from build123d import *

# Parameters (mm, degrees)
PATTERN_LINEAR_1_COUNT      = 2
PATTERN_LINEAR_1_PITCH      = 30.405591591
PATTERN_LINEAR_1_COUNT_DIR2 = 2
PATTERN_LINEAR_1_PITCH_DIR2 = 30.405591591


with BuildPart() as part:
    # 草图1 → 旋转1 (revolve)
    with BuildSketch(Plane.XY, mode=Mode.PRIVATE) as revolve_1_sk:
        with BuildLine():
            Line((0, 27), (0, 10))
            Line((0, 10), (65, 10))
            Line((65, 10), (65, 14.4))
            ThreePointArc((65, 14.4), (64.53137085, 15.53137085), (63.4, 16))
            Line((63.4, 16), (9.5, 16))
            Line((9.5, 16), (9.5, 15.5))
            Line((9.5, 15.5), (8, 15.5))
            Line((8, 15.5), (8, 27))
            Line((8, 27), (0, 27))
        make_face()
    revolve(revolve_1_sk.sketch.rotate(Axis((65, 0, 0), (-1, 0, 0)), 270), axis=Axis((65, 0, 0), (-1, 0, 0)))

    # 草图2 → 切除-旋转1 (revolve, cut)
    with BuildSketch(Plane.XY, mode=Mode.PRIVATE) as cut_revolve_1_sk:
        Polygon((0, 21.5), (0, 26), (5.1, 26), (5.1, 24.25), (8, 24.25), (8, 21.5), align=None)
    cut_revolve_1 = revolve(cut_revolve_1_sk.sketch.rotate(Axis((8, 21.5, 0), (-1, 0, 0)), 270), axis=Axis((8, 21.5, 0), (-1, 0, 0)), mode=Mode.SUBTRACT)

    # 阵列(线性)1: Cut-Revolve 1 2 × 2
    with Locations(*[Vector(0, -0.7071067811865475, 0.7071067811865477) * (i * PATTERN_LINEAR_1_PITCH) + Vector(0, -0.7071067811865477, -0.7071067811865474) * (j * PATTERN_LINEAR_1_PITCH_DIR2) for i in range(PATTERN_LINEAR_1_COUNT) for j in range(PATTERN_LINEAR_1_COUNT_DIR2) if (i, j) != (0, 0)]):
        add(cut_revolve_1, mode=Mode.SUBTRACT)


solid = part.part
Here's how the part is built. I have some questions about the finished solid (model axes, mm). A direction names the side the tool comes from. Round coordinates to 2 decimals unless told otherwise and drop trailing zeros. Loops run counter-clockwise (first coordinate to the right, second up) from the corner with the lowest first, then second, coordinate; pieces in that order, holes last.
1. Which directions (+Z, -Z, +X, -X, +Y, -Y) give clear straight access to the entire face, cutting with the end or side of a thin tool? Please do faces 4 (the face through (2.59, -17.04, -0.59)), 5 (the face through (8.74, 15.368, -2.018)), 6 (the face through (65, 10, -3)).
Answer list:
face 4: -X
face 5: none
face 6: +Z, -Z, +X, +Y, -Y
2. If I drill on line 1 along Y through (x, z) = (6.8, 0); line 2 along Z through (x, y) = (50, 0.5); line 3 along X through (y, z) = (-17.5, -6), over which ranges is the centre line in solid material (lowest first)?
Answer list:
line 1: y = -27 to -24.25, -18.75 to -10, 10 to 18.75, 24.25 to 27
line 2: z = -15.99 to -9.99, 9.99 to 15.99
line 3: x = 0 to 8
3. For P1, Ø9, axis at y = -21.5, z = 0, coming from the +X side; P2, Ø2.5, axis at y = -0.5, z = 19.5, coming from the -X side; P3, Ø12, axis at y = 0, z = 0, coming from the +X side; P4, Ø1, axis at x = 12.5, y = -12.5, coming from the -Z side, each with a flat end and sliding along its axis, tell me the tip position at first contact or that it passes through.
Answer list:
P1: stops at x = 8
P2: stops at x = 5.1
P3: passes through
P4: stops at z = -10.58
4. If we section it at A-A on z = 0: Count the separate pieces of the cut face and the enclosed holes in it, plus the area to 3 significant figures.
Answer list:
separate pieces: 4
enclosed holes: 0
area: 830 mm2
5. If we section it at D-D on z = -21.5: Write out the boundary of the cut face in (x, y), plus the area to 3 significant figures.
Answer list:
outline: (0, -16.33) - (8, -16.33) - (8, -2.75) - (5.1, -2.75) - (5.1, -4.5) - (0, -4.5) - close; (0, 4.5) - (5.1, 4.5) - (5.1, 2.75) - (8, 2.75) - (8, 16.33) - (0, 16.33) - close
area: 199 mm2
6. If we section it at C-C on x = 6: Write out the boundary of the cut face in (y, z), plus the area to 3 significant figures.
Answer list:
outline: circle Ø54 at (0, 0); hole circle Ø5.5 at (-21.5, 0); hole circle Ø20 at (0, 0); hole circle Ø5.5 at (0, -21.5); hole circle Ø5.5 at (0, 21.5); hole circle Ø5.5 at (21.5, 0)
area: 1,880 mm2
7. We'd pull the mould along Z, two halves only. Please class faces 1 (the face through (36.07, -15.62, -3.47)), 2 (the face through (0, 0, 12)), 3 (the face through (3, 0, -26)): +Z half, -Z half, draft (parallel to the pull), parting line (faces both ways), or undercut.
Answer list:
face 1: parting line
face 2: draft
face 3: undercut
